```python
from build123d import *

# Parameters (mm, degrees)
SKETCH1_R           = 100
SKETCH1_R_2         = 50
BOSS_EXTRUDE1_DEPTH = 100


with BuildPart() as part:
    # Sketch1 → Boss-Extrude1 (new body)
    with BuildSketch(Plane.XY):
        with BuildLine():
            Line((11.976047904, 199.641113693), (1675.988023952, 99.820556847))
            ThreePointArc((1675.988023952, 99.820556847), (1770, 0), (1675.988023952, -99.820556847))
            Line((1675.988023952, -99.820556847), (11.976047904, -199.641113693))
            ThreePointArc((11.976047904, -199.641113693), (-200, 0), (11.976047904, 199.641113693))
        make_face()
        Circle(SKETCH1_R, mode=Mode.SUBTRACT)
        with Locations((1670, 0)):
            Circle(SKETCH1_R_2, mode=Mode.SUBTRACT)
    extrude(amount=BOSS_EXTRUDE1_DEPTH)


solid = part.part
```
Work out the finished part from the listing and answer in its coordinate system (mm). Round coordinates to 2 decimals unless told otherwise and drop trailing zeros. Loops run counter-clockwise (first coordinate to the right, second up) from the corner with the lowest first, then second, coordinate; pieces in that order, holes last. Notation, with made-up numbers: M 86.5,40 L 133.5,40 A15 cw 133.5,49 Z; hole C 50.25,-21 d7. An arc over 180 degrees is marked long. One line per question, with ' | ' between items.
Q1. Find section D-D, the plane y = -121.5. Give the vertices of the cut face in (x, z).
Conclusion:
outline: M -158.86,0 L 1314.59,0 L 1314.59,100 L -158.86,100 Z
Q2. Consider line 1 along Y through (x, z) = (0, 32); line 2 along Y through (x, z) = (1670, 57); line 3 along X through (y, z) = (8, 27.5). Determine where each line is inside the solid, lowest interval first. Write a range as from..to.
Conclusion:
line 1: y = -200..-100, 100..200 | line 2: y = -100.18..-50, 50..100.18 | line 3: x = -199.84..-99.68, 99.68..1620.64, 1719.36..1769.68
Q3. Find section B-B, the plane z = 64. Give the vertices of the cut face in (x, y).
Conclusion:
outline: M 11.98,-199.64 L 1675.99,-99.82 A100 ccw 1675.99,99.82 L 11.98,199.64 A200 ccw long Z; hole C 0,0 d200; hole C 1670,0 d100
Q4. Find section C-C, the plane x = 230. Give the vertices of the cut face in (y, z), then the cut area to 3 significant figures.
Conclusion:
outline: M -186.56,0 L 186.56,0 L 186.56,100 L -186.56,100 Z | area: 37,300 mm2
Q5. The mould has two halves that part along Y. Classify faces 1 (the cylindrical face through (95.38, 30.04, 49.3)), 2 (the cylindrical face through (-199.948, -4.566, 49.3)), 3 (the flat face through (855.63, -149.032, 49.3)): +Y half, -Y half, draft (parallel to the pull), parting line (faces both ways), or undercut.
Conclusion:
face 1: undercut | face 2: parting line | face 3: -Y half
Q6. Each of these flat-tipped pins is pushed along its axis until it touches: pin 1 Ø5 at (y, z) = (98.5, 76.5) entering from -X; pin 2 Ø6 at (x, z) = (1485, 30.5) entering from +Y; pin 3 Ø5 at (y, z) = (38, 76.5) entering from -X. Where does it stop, or does it pass through?
Conclusion:
pin 1: stops at x = -175.45 | pin 2: stops at y = 111.46 | pin 3: stops at x = -196.82
Q7. Find section A-A, the plane y = 0. Give the vertices of the cut face in (x, z).
Conclusion:
outline: M -200,0 L -100,0 L -100,100 L -200,100 Z; M 100,0 L 1620,0 L 1620,100 L 100,100 Z; M 1720,0 L 1770,0 L 1770,100 L 1720,100 Z
